The drawing under review shows one solid part. Ordinate dimensions are in mm from its lowest x, y, z. Round coordinates to 2 decimals unless told otherwise and drop trailing zeros. Write each loop counter-clockwise with the first axis right and the second up, starting at its lowest first coordinate (ties: lowest second). Pieces come first, ordered by that corner, then holes. Notation, with made-up numbers: (46.5, 33.5) -> (83.5, 33.5) arc R19 ccw to (83.5, 53.5) -> close; hole circle Ø10 at (-12.5, 35). An arc over 180 degrees is marked (long way). Answer in a Markdown table with one row per item.
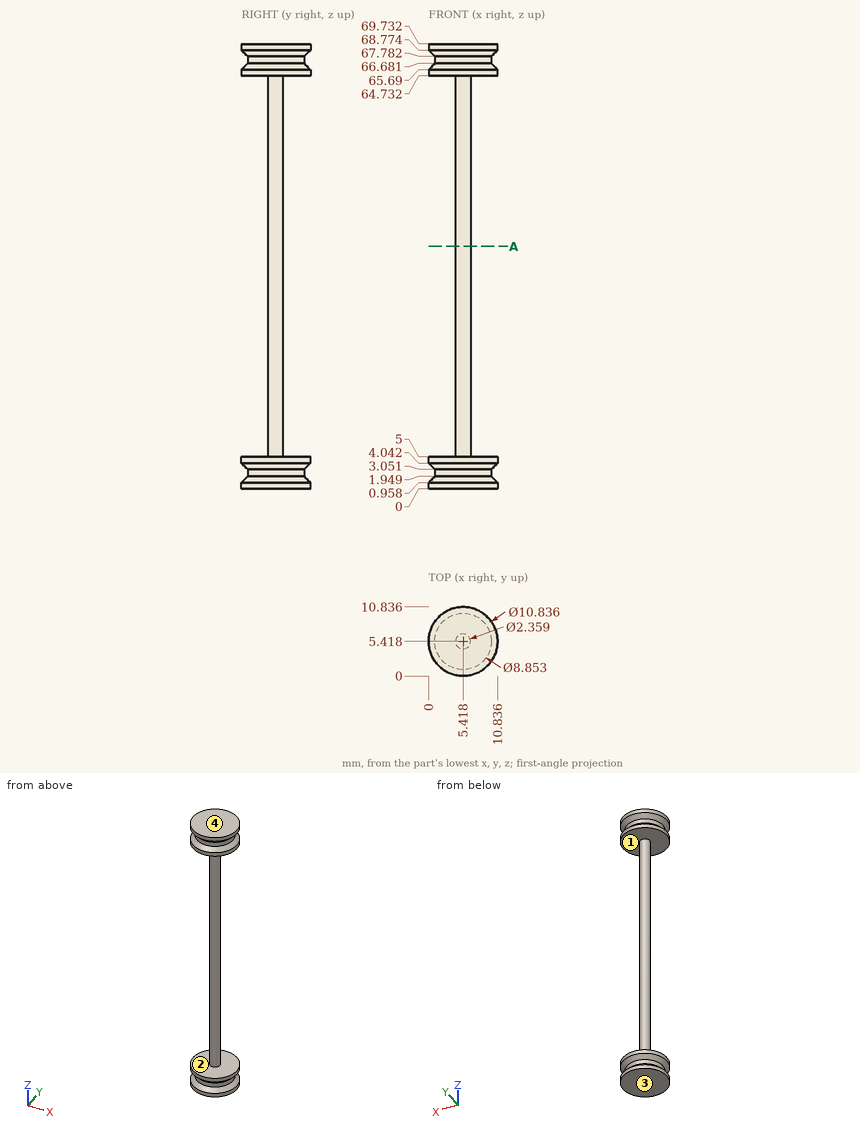
1) Clearance check with flat-ended pins moving along their axes: pin 1 Ø5 at (x, z) = (7, 53) entering from +Y; pin 2 Ø3 at (y, z) = (3, 56.5) entering from -X (1 decimal); pin 3 Ø6 at (y, z) = (6.5, 32) entering from -X; pin 4 Ø3 at (x, y) = (1.5, 7.5) entering from -Z. State where each tip first meets the part, or that it passes through.
Solved:
| item | result |
|---|---|
| pin 1 | y = 6.6 |
| pin 2 | x = 4.7 |
| pin 3 | x = 4.24 |
| pin 4 | z = 0 |
2) Mouldability with a two-part tool opening along Z and no side actions: class the marked faces 1, 2, 3 and 4 as pulls with the +Z half, pulls with the -Z half, needs draft (parallel to the pull), parting line crosses it, or undercut.
Solved:
| item | result |
|---|---|
| face 1 | undercut |
| face 2 | undercut |
| face 3 | pulls with the -Z half |
| face 4 | pulls with the +Z half |
3) Consider section A-A on z = 38. State the section outline as (x, y) points.
Solved:
| item | result |
|---|---|
| outline | circle Ø2.36 at (5.42, 5.42) |
4) For line 1 (Z direction, x = 9.25, y = 4.25); line 2 (Z direction, x = 6.25, y = 0.5) (1 decimal); line 3 (Z direction, x = 3.25, y = 1.25) (1 decimal), list the stretches that pass through material, from the lowest coordinate up. Write a range as [from, to].
Solved:
| item | result |
|---|---|
| line 1 | [0, 5], [64.73, 69.73] |
| line 2 | [0, 1.4], [3.6, 5], [64.7, 66.1], [68.3, 69.7] |
| line 3 | [0, 1.7], [3.3, 5], [64.7, 66.4], [68.1, 69.7] |
